from build123d import *

# Parameters (mm, degrees)
SKETCH1_W                = 50
SKETCH1_H                = 100
BOSS_EXTRUDE1_DEPTH      = 5
CUT_EXTRUDE1_DEPTH       = 10
SKETCH3_R                = 5
CUT_EXTRUDE2_DEPTH       = 10
BOSS_EXTRUDE2_DEPTH      = 100
BOSS_EXTRUDE2_DEPTH_BACK = 5
SKETCH4_W                = 50
SKETCH4_H                = 5
CUT_EXTRUDE3_DEPTH       = 80


with BuildPart() as part:
    # Sketch1 → Boss-Extrude1 (new body)
    with BuildSketch(Plane.XY):
        Rectangle(SKETCH1_W, SKETCH1_H)
    extrude(amount=BOSS_EXTRUDE1_DEPTH)

    # Sketch2 → Cut-Extrude1 (cut)
    with BuildSketch(Plane.XY.offset(5)):
        with BuildLine():
            Line((-14.5, -43.655057898), (-15.5, -43.655057898))
            ThreePointArc((-15.5, -43.655057898), (-17.267766953, -42.922824851), (-18, -41.155057898))
            Line((-18, -41.155057898), (-18, 28.844942102))
            ThreePointArc((-18, 28.844942102), (-17.267766953, 30.612709055), (-15.5, 31.344942102))
            Line((-15.5, 31.344942102), (-14.5, 31.344942102))
            ThreePointArc((-14.5, 31.344942102), (-12.732233047, 30.612709055), (-12, 28.844942102))
            Line((-12, 28.844942102), (-12, -41.155057898))
            ThreePointArc((-12, -41.155057898), (-12.732233047, -42.922824851), (-14.5, -43.655057898))
        make_face()
        with BuildLine():
            Line((15.5, -43.655057898), (14.5, -43.655057898))
            ThreePointArc((14.5, -43.655057898), (12.732233047, -42.922824851), (12, -41.155057898))
            Line((12, -41.155057898), (12, 28.844942102))
            ThreePointArc((12, 28.844942102), (12.732233047, 30.612709055), (14.5, 31.344942102))
            Line((14.5, 31.344942102), (15.5, 31.344942102))
            ThreePointArc((15.5, 31.344942102), (17.267766953, 30.612709055), (18, 28.844942102))
            Line((18, 28.844942102), (18, -41.155057898))
            ThreePointArc((18, -41.155057898), (17.267766953, -42.922824851), (15.5, -43.655057898))
        make_face()
    extrude(amount=-CUT_EXTRUDE1_DEPTH, mode=Mode.SUBTRACT)

    # Sketch3 → Cut-Extrude2 (cut)
    with BuildSketch(Plane.XY.offset(5)):
        Circle(SKETCH3_R)
    extrude(amount=-CUT_EXTRUDE2_DEPTH, mode=Mode.SUBTRACT)

    # Sketch4 → Boss-Extrude2 (add, two sides: drawn at the far end of the back side and taken through both)
    with BuildSketch(Plane(origin=(0, 0, 0), x_dir=(-1, 0, 0), z_dir=(0, 0, -1)).offset(-BOSS_EXTRUDE2_DEPTH_BACK)):
        with Locations((0, 52.5)):
            Rectangle(SKETCH4_W, SKETCH4_H)
    extrude(amount=BOSS_EXTRUDE2_DEPTH + BOSS_EXTRUDE2_DEPTH_BACK)

    # Sketch5 → Cut-Extrude3 (cut)
    with BuildSketch(Plane.XZ.offset(-50)):
        with BuildLine():
            Line((-0.473985761, -94.252877225), (-1.473985761, -94.252877225))
            ThreePointArc((-1.473985761, -94.252877225), (-4.655966276, -92.934857741), (-5.973985761, -89.752877225))
            Line((-5.973985761, -89.752877225), (-5.973985761, -13.752877225))
            ThreePointArc((-5.973985761, -13.752877225), (-4.655966276, -10.57089671), (-1.473985761, -9.252877225))
            Line((-1.473985761, -9.252877225), (-0.473985761, -9.252877225))
            ThreePointArc((-0.473985761, -9.252877225), (2.707994755, -10.57089671), (4.026014239, -13.752877225))
            Line((4.026014239, -13.752877225), (4.026014239, -89.752877225))
            ThreePointArc((4.026014239, -89.752877225), (2.707994755, -92.934857741), (-0.473985761, -94.252877225))
        make_face()
    extrude(amount=-CUT_EXTRUDE3_DEPTH, mode=Mode.SUBTRACT)


solid = part.part
Can you work these out from the model? Positions are in its coordinate system, mm. A direction names the side the tool comes from. Coordinates: 2 decimals unless noted, no trailing zeros. Write each loop counter-clockwise with the first axis right and the second up, starting at its lowest first coordinate (ties: lowest second). Pieces come first, ordered by that corner, then holes. Notation, with made-up numbers: (63, 47) -> (93, 47) arc R21 ccw to (93, 61) -> close; hole circle Ø4 at (75, 88.25). An arc over 180 degrees is marked (long way). Write item = value, one per line.
(1) Imagine slicing it at A-A (y = 0). Please give me the cut outline in (x, z), and give its area (3 significant figures).
Verdict:
outline = (-25, 0) -> (-18, 0) -> (-18, 5) -> (-25, 5) -> close; (-12, 0) -> (-5, 0) -> (-5, 5) -> (-12, 5) -> close; (5, 0) -> (12, 0) -> (12, 5) -> (5, 5) -> close; (18, 0) -> (25, 0) -> (25, 5) -> (18, 5) -> close
area = 140 mm^2
(2) If I drill on probe 1 along Y at (x, z) = (0, 2.7); probe 2 along Z at (x, y) = (19.5, 8); probe 3 along Y at (x, z) = (-11, -23), over which ranges is the centre line in solid material (lowest first)?
Verdict:
probe_1 = -50 to -5, 5 to 55
probe_2 = 0 to 5
probe_3 = 50 to 55
(3) Thinking about a two-plate mould opening in Y: for faces 1 (the face through (0, -50, 2)), 2 (the face through (-6, 1, 0)), 3 (the face through (-12, -6, 3)), which applies, +Y half, -Y half, draft (parallel to the pull), parting line (faces both ways), or undercut?
Verdict:
face_1 = -Y half
face_2 = draft
face_3 = undercut
(4) For pin 1 (1 mm diameter, centred on x = -1, z = -11, fed in from -Y); pin 2 (4 mm diameter, centred on x = 11.5, z = -79, fed in from -Y); pin 3 (25 mm diameter, centred on x = 4.5, y = -24, fed in from -Z), each with a flat end and sliding along its axis, tell me the tip position at first contact or that it passes through.
Verdict:
pin_1 = through
pin_2 = 50
pin_3 = 0
(5) Imagine slicing it at B-B (z = -39). Please give me the cut outline in (x, y), and give its area (3 significant figures).
Verdict:
outline = (-25, 50) -> (-5.97, 50) -> (-5.97, 55) -> (-25, 55) -> close; (4.03, 50) -> (25, 50) -> (25, 55) -> (4.03, 55) -> close
area = 200 mm^2
(6) On a 3-axis mill with a long thin cutter (end or side, diameter ignored), from which of +Z, -Z, +X, -X, +Y, -Y can I reach the whole of each face in a straight line? I mean faces 4 (the face through (-25, 26, 3)), 5 (the face through (12.75, -42.94, 2.54)), 6 (the face through (-5.974, 52, -52)). Say none if no direction works.
Verdict:
face_4 = +Z, -Z, -X, +Y, -Y
face_5 = +Z, -Z
face_6 = +Y, -Y
(7) Imagine slicing it at D-D (x = 9.5). Please give me the cut outline in (y, z).
Verdict:
outline = (-50, 0) -> (50, 0) -> (50, -100) -> (55, -100) -> (55, 5) -> (-50, 5) -> close
(8) Imagine slicing it at C-C (y = -31). Please give me the cut outline in (x, z).
Verdict:
outline = (-25, 0) -> (-18, 0) -> (-18, 5) -> (-25, 5) -> close; (-12, 0) -> (12, 0) -> (12, 5) -> (-12, 5) -> close; (18, 0) -> (25, 0) -> (25, 5) -> (18, 5) -> close
